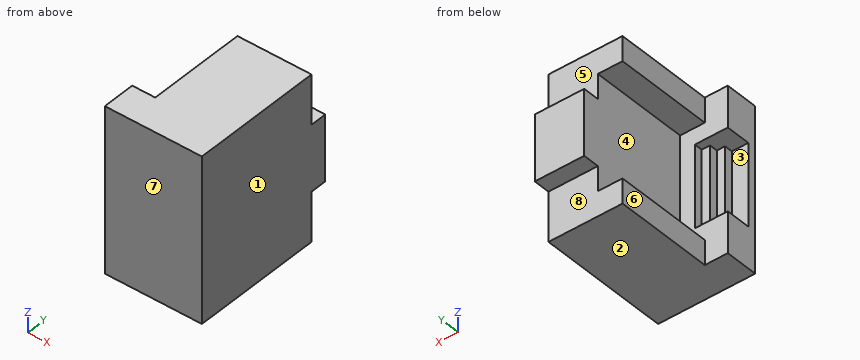
from build123d import *

# Parameters (mm, degrees)
BASE_BLOCK_DEPTH          = 1000
SIDE_BOSS_A_SKETCH_W      = 150
SIDE_BOSS_A_SKETCH_H      = 600
SIDE_BOSS_A_DEPTH         = 150
SIDE_BOSS_B_SKETCH_W      = 150
SIDE_BOSS_B_SKETCH_H      = 600
SIDE_BOSS_B_DEPTH         = 150
CORNER_BOSS_DEPTH         = 100
TOP_STEP_CUT_DEPTH        = 150
TOP_GROOVE_CUT_DEPTH      = 1450.689621954
TOP_GROOVE_CUT_DEPTH_BACK = 100
GROOVE_NOTCH_SKETCH_W     = 500
GROOVE_NOTCH_SKETCH_H     = 50
GROOVE_NOTCH_CUT_DEPTH    = 50
GROOVE_INFILL_BOSS_DEPTH  = 50


with BuildPart() as part:
    # Base Profile Sketch → Base Block (new body)
    with BuildSketch(Plane.XY):
        Polygon((0, 0), (540, 0), (540, 800), (240, 800), (240, 200), (0, 200), align=None)
    extrude(amount=BASE_BLOCK_DEPTH)

    # Side Boss A Sketch → Side Boss A (add)
    with BuildSketch(Plane(origin=(0, 0, 0), x_dir=(-1, 0, 0), z_dir=(0, 0, -1))):
        with Locations((-165, 500)):
            Rectangle(SIDE_BOSS_A_SKETCH_W, SIDE_BOSS_A_SKETCH_H)
    extrude(amount=-SIDE_BOSS_A_DEPTH)

    # Side Boss B Sketch → Side Boss B (add)
    with BuildSketch(Plane.XY.offset(1000)):
        with Locations((165, 500)):
            Rectangle(SIDE_BOSS_B_SKETCH_W, SIDE_BOSS_B_SKETCH_H)
    extrude(amount=-SIDE_BOSS_B_DEPTH)

    # Corner Boss Sketch → Corner Boss (add)
    with BuildSketch(Plane(origin=(0, 800, 0), x_dir=(1, 0, 0), z_dir=(0, 1, 0))):
        Polygon((540, -500), (540, -300), (240, -300), (240, -700), (540, -700), align=None)
    extrude(amount=CORNER_BOSS_DEPTH)

    # Top Step Cut Sketch → Top Step Cut (cut)
    with BuildSketch(Plane.ZY):
        Polygon((500, 200), (250, 200), (250, 150), (750, 150), (750, 200), align=None)
    extrude(amount=-TOP_STEP_CUT_DEPTH, mode=Mode.SUBTRACT)

    # Top Groove Sketch → Top Groove Cut (cut, two sides: drawn at the far end of the back side and taken through both)
    with BuildSketch(Plane.ZY.offset(-TOP_GROOVE_CUT_DEPTH_BACK)):
        Polygon((250, 2281.32034356), (250, 150), (250, 100), (750, 100), (750, 150), (750, 2281.32034356), (750, 6543.961030679), (250, 6543.961030679), align=None)
    extrude(amount=TOP_GROOVE_CUT_DEPTH + TOP_GROOVE_CUT_DEPTH_BACK, mode=Mode.SUBTRACT)

    # Groove Notch Sketch → Groove Notch Cut (cut)
    with BuildSketch(Plane.ZY):
        with Locations((500, 75)):
            Rectangle(GROOVE_NOTCH_SKETCH_W, GROOVE_NOTCH_SKETCH_H)
    extrude(amount=-GROOVE_NOTCH_CUT_DEPTH, mode=Mode.SUBTRACT)

    # Groove Infill Sketch → Groove Infill Boss (add)
    with BuildSketch(Plane.ZY):
        Polygon((0, 200), (0, 0), (1000, 0), (1000, 200), (750, 200), (750, 50), (250, 50), (250, 200), align=None)
    extrude(amount=GROOVE_INFILL_BOSS_DEPTH)


solid = part.part
For this review, take the finished solid that the model builds, in its own axes (mm). Face numbers are marked on the shaded views. A direction names the side the tool comes from. Coordinates: 2 decimals unless noted, no trailing zeros. Loops run counter-clockwise (first coordinate to the right, second up) from the corner with the lowest first, then second, coordinate; pieces in that order, holes last. Notation, with made-up numbers: (-19.75, 61.25) - (17.25, 61.25) arc R17 cw to (17.25, 77.25) - close; hole circle Ø3 at (17, -22.75). An arc over 180 degrees is marked (long way). Use a Markdown table: item, result. Add a question column.
Item 1: For line 1 (Z direction, x = 201.5, y = 476); line 2 (Z direction, x = 12, y = 191); line 3 (Y direction, x = 435, z = 954.5), list the stretches that pass through material, from the lowest coordinate up.
Item 2: Insertion check: pin 1 Ø10 at (x, z) = (262, 171) entering from -Y; pin 2 Ø3 at (x, z) = (137.5, 797) entering from +Y; pin 3 Ø25 at (x, z) = (82, 403) entering from +Y; pin 4 Ø2 at (y, z) = (447.5, 246) entering from -X. Each pin has a flat end and moves straight along its axis. Give the tip position at first contact, or say it passes through.
Item 3: We need section A-A (x = 456). Give the boundary of the cut face in (y, z), and give its area (3 significant figures).
Item 4: Tool access review of the marked faces 4, 5, 6, 7 and 8: name each direction out of +Z, -Z, +X, -X, +Y, -Y from which nothing blocks a thin tool from reaching the whole face with its end or side.
Item 5: We need section D-D (z = 196.5). Give the boundary of the cut face in (x, y).
Item 6: Mouldability with a two-part tool opening along Z and no side actions: class the marked faces 1, 2 and 3 as pulls with the +Z half, pulls with the -Z half, needs draft (parallel to the pull), parting line crosses it, or undercut.
Item 7: We need section C-C (z = 611). Give the boundary of the cut face in (x, y).
Item 8: We need section B-B (y = 287.5). Give the boundary of the cut face in (x, z), and give its area (3 significant figures).
Results list:
| question | item | result |
|---|---|---|
| 1 | line 1 | z = 0 to 150, 850 to 1000 |
| 1 | line 2 | z = 0 to 250, 750 to 1000 |
| 1 | line 3 | y = 0 to 800 |
| 2 | pin 1 | stops at y = 0 |
| 2 | pin 2 | stops at y = 200 |
| 2 | pin 3 | stops at y = 100 |
| 2 | pin 4 | stops at x = 240 |
| 3 | outline | (0, 0) - (800, 0) - (800, 300) - (900, 300) - (900, 700) - (800, 700) - (800, 1000) - (0, 1000) - close |
| 3 | area | 840,000 mm^2 |
| 4 | face 4 | -X, +Y |
| 4 | face 5 | +Z, +X, -X, +Y |
| 4 | face 6 | +Z, -Z, -X, +Y |
| 4 | face 7 | +Z, -Z, +X, -X, -Y |
| 4 | face 8 | -Z, +X, -X, +Y |
| 5 | outline | (-50, 0) - (540, 0) - (540, 800) - (240, 800) - (240, 200) - (-50, 200) - close |
| 6 | face 1 | needs draft |
| 6 | face 2 | pulls with the -Z half |
| 6 | face 3 | undercut |
| 7 | outline | (-50, 0) - (540, 0) - (540, 900) - (240, 900) - (240, 200) - (150, 200) - (150, 150) - (100, 150) - (100, 100) - (50, 100) - (50, 50) - (-50, 50) - close |
| 8 | outline | (90, 0) - (540, 0) - (540, 1000) - (90, 1000) - (90, 850) - (240, 850) - (240, 150) - (90, 150) - close |
| 8 | area | 345,000 mm^2 |
